For this review, use the dimensioned drawing (mm, ordinates from the lowest corner) and the shaded views. A direction names the side the tool comes from. Round coordinates to 2 decimals unless told otherwise and drop trailing zeros. Order: outer loops, then holes, each group sorted by start corner. A loop starts at its lowest first (then second) coordinate and runs counter-clockwise, first axis right, second up. Notation, with made-up numbers: (58.25, 26.5) -> (97.25, 26.5) arc R28 ccw to (97.25, 65.5) -> close; hole circle Ø6 at (85.25, -5.5). An arc over 180 degrees is marked (long way). Use a Markdown table: item, result. Add a question column.
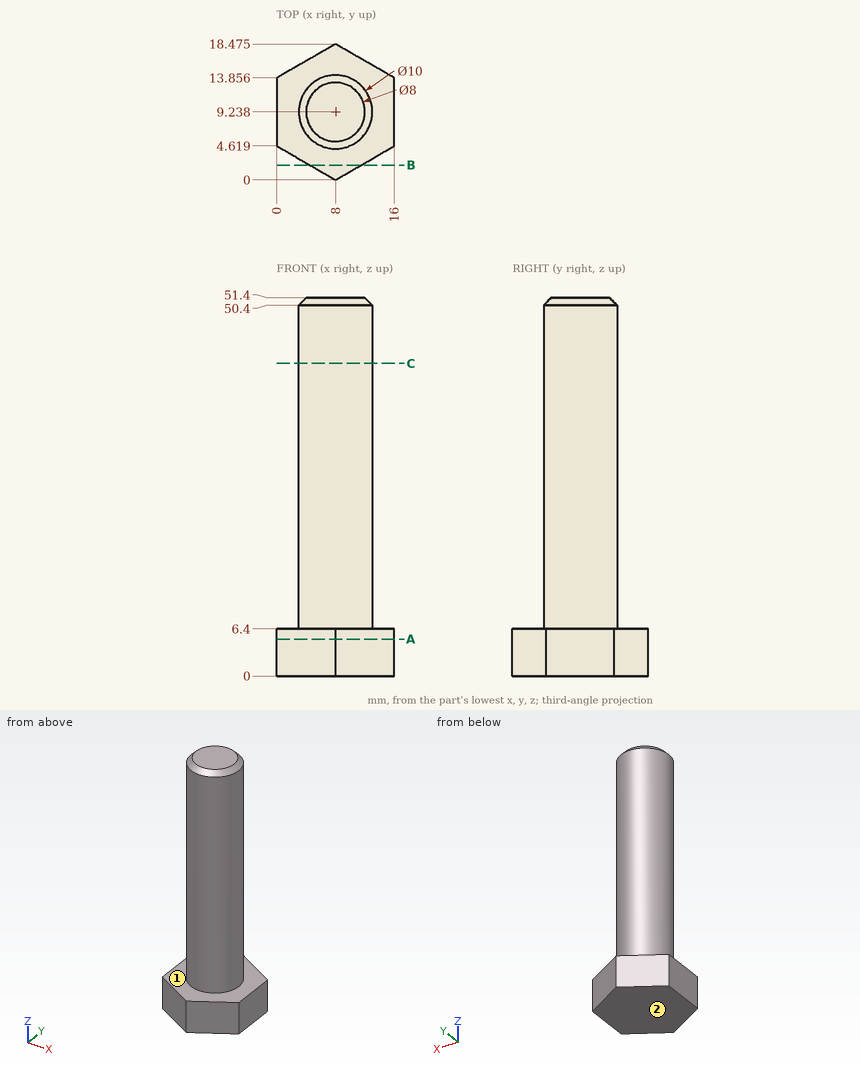
Q1. Machinability: for the marked faces 1 and 2, which of the approach directions +Z, -Z, +X, -X, +Y, -Y give a long, thin tool a straight path to every point of the face, cutting with its end or side? Answer none if there is none.
Q2. Add section C-C (z = 42.5). Write out the cut boundary in (x, y).
Q3. Add section A-A (z = 5). Write out the cut boundary in (x, y) (1 decimal).
Q4. Insertion check: pin 1 (1.5 mm diameter, centred on x = 4, z = 26.5, fed in from +Y); pin 2 (2 mm diameter, centred on x = 5.5, z = 16, fed in from +Y); pin 3 (8 mm diameter, centred on x = 2, y = 10, fed in from +Z); pin 4 (5 mm diameter, centred on y = 5.5, z = 38, fed in from +X) (1 decimal). Each pin has a flat end and moves straight along its axis. Give the tip position at first contact, or say it passes through.
Q5. Add section B-B (y = 2). Write out the cut boundary in (x, z).
Q6. Wall thickness on line 1 (Z direction, x = 2, y = 12); line 2 (X direction, y = 9.5, z = 29); line 3 (X direction, y = 6.25, z = 36): over which ranges is each line inside the solid? List them lowest first. Write a range as [from, to].
Report:
| question | item | result |
|---|---|---|
| 1 | face 1 | +Z |
| 1 | face 2 | -Z, +X, -X, +Y, -Y |
| 2 | outline | circle Ø10 at (8, 9.24) |
| 3 | outline | (0, 4.6) -> (8, 0) -> (16, 4.6) -> (16, 13.9) -> (8, 18.5) -> (0, 13.9) -> close |
| 4 | pin 1 | stops at y = 13.04 |
| 4 | pin 2 | stops at y = 14.01 |
| 4 | pin 3 | stops at z = 51.4 |
| 4 | pin 4 | stops at x = 12.8 |
| 5 | outline | (4.54, 0) -> (11.46, 0) -> (11.46, 6.4) -> (4.54, 6.4) -> close |
| 6 | line 1 | z = [0, 6.4] |
| 6 | line 2 | x = [3.01, 12.99] |
| 6 | line 3 | x = [3.99, 12.01] |
